Check sheet for the modelled part. Datum: model origin and axes. Units: mm. Coordinates: 2 decimals unless noted, no trailing zeros. Loops run counter-clockwise (first coordinate to the right, second up) from the corner with the lowest first, then second, coordinate; pieces in that order, holes last. Notation, with made-up numbers: (44.5, 35) - (91.5, 35) arc R18 ccw to (91.5, 42) - close; hole circle Ø4 at (28.25, -26.75). An arc over 180 degrees is marked (long way). Write each question's results on one line, items separated by ' | '. Start each with the question number.
1. Cross-section at B-B (x = 22.5). Give the number of separate pieces and of enclosed holes in the cut face, and give its area (3 significant figures).
2. Gauge pin test, flat end, axial feed: P1, Ø5.5, axis at x = 22.5, z = -41.5, coming from the +Y side. Record the tip position at first contact, or that the pin passes through.
3. Draft check along Z on faces 1 (the face through (-27.32, -7.86, -47.19)), 2 (the face through (27.44, -3.95, 42.58)), 3 (the face through (25.743, -3.944, 35.479)). Enter one of: released by +Z, released by -Z, zero draft, split by the parting line, or undercut.
4. Thickness scan on line 1 (X direction, y = -4.5, z = -41.5); line 2 (Z direction, x = 24.5, y = -7); line 3 (Z direction, x = 22.5, y = -3.75). Record the ranges inside material, lowest first. Write a range as [from, to].
5. Cross-section at A-A (y = -2.5). Record the cut outline in (x, z).
```python
from build123d import *

# Parameters (mm, degrees)
SKETCH1_W                  = 60
SKETCH1_H                  = 95
BOSS_EXTRUDE1_DEPTH        = 8
F_6_8_6_8_DIAMETER_HOLE1_D = 6.8
FILLET1_R                  = 8.5
CHAMFER1_SIZE              = 0.5


with BuildPart() as part:
    # Sketch1 → Boss-Extrude1 (new body)
    with BuildSketch(Plane.XZ.offset(8)):
        with Locations((0, -2.5)):
            Rectangle(SKETCH1_W, SKETCH1_H)
    extrude(amount=-BOSS_EXTRUDE1_DEPTH)

    # Ø6.8 (6.8) Diameter Hole1 (through all)
    with Locations(Plane(origin=(0, -8, 0), x_dir=(-1, 0, 0), z_dir=(0, -1, 0))):
        with Locations((22.5, 41.5), (-22.5, 41.5), (-22.5, -36.5), (22.5, -36.5)):
            Hole(F_6_8_6_8_DIAMETER_HOLE1_D / 2)

    # Fillet1
    fillet1_edges = [part.edges().sort_by_distance(p)[0] for p in [
        (-30, -4, 45),
        (30, -4, 45),
        (30, -4, -50),
        (-30, -4, -50),
    ]]
    fillet(fillet1_edges, radius=FILLET1_R)

    # Chamfer1
    chamfer1_edges = [part.edges().sort_by_distance(p)[0] for p in [
        (0, -8, -50),
        (0, 0, -50),
        (-30, -8, -2.5),
        (30, -8, -2.5),
        (0, -8, 45),
        (-27.51040764, -8, 42.51040764),
        (-27.51040764, -8, -47.51040764),
        (27.51040764, -8, 42.51040764),
        (27.51040764, -8, -47.51040764),
        (30, 0, -2.5),
        (-30, 0, -2.5),
        (0, 0, 45),
        (-27.51040764, 0, 42.51040764),
        (-27.51040764, 0, -47.51040764),
        (27.51040764, 0, 42.51040764),
        (27.51040764, 0, -47.51040764),
    ]]
    chamfer(chamfer1_edges, length=CHAMFER1_SIZE)


solid = part.part
```
Established:
1) separate pieces: 3 | enclosed holes: 0 | area: 650 mm^2
2) P1: through
3) face 1: released by -Z | face 2: released by +Z | face 3: undercut
4) line 1: [-30, -25.9], [-19.1, 19.1], [25.9, 30] | line 2: [-49.45, -44.25], [-38.75, 33.75], [39.25, 44.45] | line 3: [-49.94, -44.9], [-38.1, 33.1], [39.9, 44.94]
5) outline: (-30, -41.5) arc R8.5 ccw to (-21.5, -50) - (21.5, -50) arc R8.5 ccw to (30, -41.5) - (30, 36.5) arc R8.5 ccw to (21.5, 45) - (-21.5, 45) arc R8.5 ccw to (-30, 36.5) - close; hole circle Ø6.8 at (-22.5, -41.5); hole circle Ø6.8 at (-22.5, 36.5); hole circle Ø6.8 at (22.5, -41.5); hole circle Ø6.8 at (22.5, 36.5)
